from build123d import *

# Parameters (mm, degrees)
SKETCH1_R           = 10
BOSS_EXTRUDE1_DEPTH = 374
CUT_EXTRUDE1_START  = -8
SKETCH_2_2_W        = 44.374102045
SKETCH_2_2_H        = 48.77153558
SKETCH_2_2_W_2      = 193.002207495
SKETCH_2_2_H_2      = 56.618631092
CUT_EXTRUDE1_DEPTH  = 20
CUT_EXTRUDE2_START  = 8
SKETCH_2_2_2_W      = 44.374102045
SKETCH_2_2_2_H      = 48.77153558
SKETCH_2_2_2_W_2    = 193.002207495
SKETCH_2_2_2_H_2    = 56.618631092
CUT_EXTRUDE2_DEPTH  = 20


with BuildPart() as part:
    # Sketch1 → Boss-Extrude1 (new body)
    with BuildSketch(Plane(origin=(0, 0, 0), x_dir=(0, 0, -1), z_dir=(1, 0, 0))):
        Circle(SKETCH1_R)
    extrude(amount=BOSS_EXTRUDE1_DEPTH)

    # Sketch 2_2 → Cut-Extrude1 (cut)
    with BuildSketch(Plane.XY.offset(CUT_EXTRUDE1_START)):
        with Locations((10.312948977, 5.596733591)):
            Rectangle(SKETCH_2_2_W, SKETCH_2_2_H)
        with Locations((438.001103747, 0.32564759)):
            Rectangle(SKETCH_2_2_W_2, SKETCH_2_2_H_2)
    extrude(amount=-CUT_EXTRUDE1_DEPTH, mode=Mode.SUBTRACT)

    # Sketch 2_2 2 → Cut-Extrude2 (cut)
    with BuildSketch(Plane.XY.offset(CUT_EXTRUDE2_START)):
        with Locations((10.312948977, 5.596733591)):
            Rectangle(SKETCH_2_2_2_W, SKETCH_2_2_2_H)
        with Locations((438.001103747, 0.32564759)):
            Rectangle(SKETCH_2_2_2_W_2, SKETCH_2_2_2_H_2)
    extrude(amount=CUT_EXTRUDE2_DEPTH, mode=Mode.SUBTRACT)


solid = part.part
Input: part model. Units: mm. Frame: model coordinates. A direction names the side the tool comes from. Coordinates: 2 decimals unless noted, no trailing zeros. Loops run counter-clockwise (first coordinate to the right, second up) from the corner with the lowest first, then second, coordinate; pieces in that order, holes last.
(1) Section B-B on x = 23. Return the cut outline in (y, z), then the cut area to 3 significant figures.
(2) Material intervals for probe 1 along Z at (x, y) = (304, -0.75); probe 2 along Z at (x, y) = (169, 3.25); probe 3 along Y at (x, z) = (354, 6.5), sorted ascending.
(3) Section A-A on y = 0. Return the cut outline in (x, z), then the cut area to 3 significant figures.
(4) Section C-C on z = 4.5. Return the cut outline in (x, y).
(5) Section D-D on x = 326. Return the cut outline in (y, z), then the cut area to 3 significant figures.
(6) Set-up query: faces 1 (the face through (0, 0, 0)), 2 (the face through (16, 0, -8)), 3 (the face through (358, 0, -8)), 4 (the face through (16, 0, 8)), 5 (the face through (358, 0, 8)). Return all of +Z, -Z, +X, -X, +Y, -Y with unobstructed straight access to the full face (end or side cutting, diameter ignored); none if empty.
(7) First-contact query: pin 1 Ø0.6 at (y, z) = (1.5, -9) entering from +X; pin 2 Ø9.5 at (x, y) = (354, 3) entering from +Z; pin 3 Ø1.6 at (y, z) = (1, 9.5) entering from -X. Flat tips, straight axial feed; report the tip coordinate or a pass-through.
Data:
1. outline: (-6, -8) - (6, -8) arc R10 ccw to (6, 8) - (-6, 8) arc R10 ccw to start
1. area: 281 mm2
2. probe 1: z = -9.97 to 9.97
2. probe 2: z = -9.46 to 9.46
2. probe 3: y = -7.6 to 7.6
3. outline: (0, -8) - (32.5, -8) - (32.5, -10) - (341.5, -10) - (341.5, -8) - (374, -8) - (374, 8) - (341.5, 8) - (341.5, 10) - (32.5, 10) - (32.5, 8) - (0, 8) - close
3. area: 7,220 mm2
4. outline: (0, -8.93) - (374, -8.93) - (374, 8.93) - (0, 8.93) - close
5. outline: circle Ø20 at (0, 0)
5. area: 314 mm2
6. face 1: +Z, -Z, -X, +Y, -Y
6. face 2: -Z, -X, +Y, -Y
6. face 3: -Z, +X, +Y, -Y
6. face 4: +Z, -X, +Y, -Y
6. face 5: +Z, +X, +Y, -Y
7. pin 1: stops at x = 341.5
7. pin 2: stops at z = 8
7. pin 3: stops at x = 32.5
